Can you work these out from the model? Positions are in its coordinate system, mm. A direction names the side the tool comes from. Round coordinates to 2 decimals unless told otherwise and drop trailing zeros. Loops run counter-clockwise (first coordinate to the right, second up) from the corner with the lowest first, then second, coordinate; pieces in that order, holes last. Notation, with made-up numbers: M -3.75,-10.5 L 3.25,-10.5 A32 ccw 3.25,20.5 Z; hole C 43.25,84.5 d5. An arc over 180 degrees is marked long. Use a Markdown table: item, result. Add a question column.
```python
from build123d import *

# Parameters (mm, degrees)
SKETCH1_W           = 450
SKETCH1_H           = 600
BOSS_EXTRUDE1_DEPTH = 400
CUT_EXTRUDE1_DEPTH  = 2400
SKETCH4_W           = 648.804514889
SKETCH4_H           = 183.272574448
CUT_EXTRUDE2_DEPTH  = 40
SKETCH5_R           = 100
BOSS_EXTRUDE2_DEPTH = 20


with BuildPart() as part:
    # Sketch1 → Boss-Extrude1 (new body)
    with BuildSketch(Plane(origin=(0, 0, 0), x_dir=(0, 0, -1), z_dir=(1, 0, 0))):
        Rectangle(SKETCH1_W, SKETCH1_H)
    extrude(amount=BOSS_EXTRUDE1_DEPTH)

    # Sketch2 → Cut-Extrude1 (cut)
    with BuildSketch(Plane.XY.offset(225)):
        Polygon((200, 300), (200, -120), (400, -230), (400, 300), align=None)
    extrude(amount=-CUT_EXTRUDE1_DEPTH, mode=Mode.SUBTRACT)

    # Sketch4 → Cut-Extrude2 (cut)
    with BuildSketch(Plane(origin=(400, 0, 0), x_dir=(0, 0, -1), z_dir=(1, 0, 0))):
        with Locations((-2.450168107, -263.148054755)):
            Rectangle(SKETCH4_W, SKETCH4_H)
    extrude(amount=-CUT_EXTRUDE2_DEPTH, mode=Mode.SUBTRACT)

    # Sketch5 → Boss-Extrude2 (add)
    with BuildSketch(Plane(origin=(200, 0, 0), x_dir=(0, 0, -1), z_dir=(1, 0, 0))):
        with Locations(Location((0, 150, 0), (0, 0, 270))):
            Circle(SKETCH5_R)
    extrude(amount=BOSS_EXTRUDE2_DEPTH)


solid = part.part
```
(1) Thinking about a two-plate mould opening in Y: for faces 4 (the face through (0, 4, 3)), 5 (the face through (177, -300, 3)), 6 (the face through (209.86, 223.704, -67.585)), which applies, released by +Y, released by -Y, zero draft, split by the parting line, or undercut?
(2) Suppose I cut it at B-B on y = 150. List the corners of the cut face in (x, z) for me, and give its area (3 significant figures).
(3) If I drill on probe 1 along Y at (x, z) = (218, 57.5); probe 2 along X at (y, z) = (-9, 179); probe 3 along Y at (x, z) = (207.5, 14.5) (3 decimals), over which ranges is the centre line in solid material (lowest first)? Write a range as [from, to].
(4) Suppose I cut it at D-D on z = 178. List the corners of the cut face in (x, y) for me, and give its area (3 significant figures).
(5) Suppose I cut it at A-A on z = 0. List the corners of the cut face in (x, y) for me.
(6) On a 3-axis mill with a long thin cutter (end or side, diameter ignored), from which of +Z, -Z, +X, -X, +Y, -Y can I reach the whole of each face in a straight line? I mean faces 1 (the face through (360, -253, 3)), 2 (the face through (200, 46, 3)), 3 (the face through (220, 151, -1)). Say none if no direction works.
(7) Suppose I cut it at C-C on x = 284.5. List the corners of the cut face in (y, z) for me (3 decimals), and give its area (3 significant figures).
(8) I'm going to push a flat-ended pin straight in: pin 1 (4 mm diameter, centred on y = -76, z = -147.5, fed in from +X). Where does the tip first touch, or does it pass through?
Results below:
| question | item | result |
|---|---|---|
| 1 | face 4 | zero draft |
| 1 | face 5 | released by -Y |
| 1 | face 6 | undercut |
| 2 | outline | M 0,-225 L 200,-225 L 200,-100 L 220,-100 L 220,100 L 200,100 L 200,225 L 0,225 Z |
| 2 | area | 94,000 mm² |
| 3 | probe 1 | y = [-300, -129.9], [68.18, 231.82] |
| 3 | probe 2 | x = [0, 200] |
| 3 | probe 3 | y = [-300, -124.125], [51.057, 248.943] |
| 4 | outline | M 0,-300 L 360,-300 L 360,-208 L 200,-120 L 200,300 L 0,300 Z |
| 4 | area | 142,000 mm² |
| 5 | outline | M 0,-300 L 360,-300 L 360,-208 L 200,-120 L 200,50 L 220,50 L 220,250 L 200,250 L 200,300 L 0,300 Z |
| 6 | face 1 | +Z, -Z, +X, +Y, -Y |
| 6 | face 2 | +X |
| 6 | face 3 | +Z, -Z, +X, +Y |
| 7 | outline | M -300,-225 L -166.475,-225 L -166.475,225 L -300,225 Z |
| 7 | area | 60,100 mm² |
| 8 | pin 1 | stops at x = 200 |
